Source: CAD feature listing. Evaluate the final solid. Frame: model axes, mm. Coordinates: 2 decimals unless noted, no trailing zeros. Loops run counter-clockwise (first coordinate to the right, second up) from the corner with the lowest first, then second, coordinate; pieces in that order, holes last.
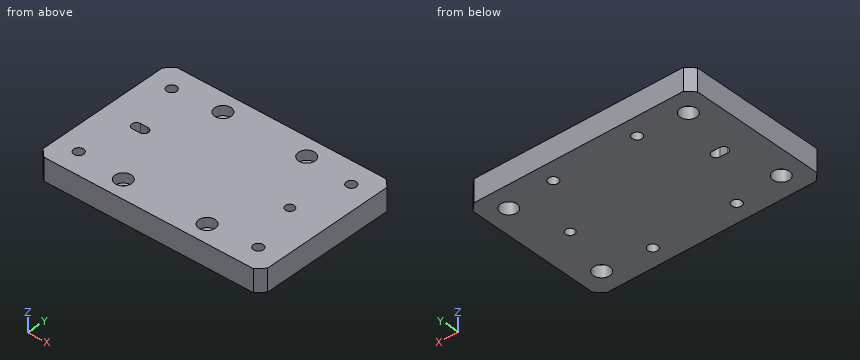
from build123d import *

# Parameters (mm, degrees)
SKETCH_1_W                   = 150
SKETCH_1_H                   = 100
EXTRUDE_1_DEPTH              = 7.5
HOLE_WIZARD_M6_1_D           = 6.6
HOLE_WIZARD_M6_1_CBORE_D     = 11
HOLE_WIZARD_M6_1_CBORE_DEPTH = 6.4
CHAMFER_1_SIZE               = 5
HOLE_WIZARD_M6_2_D           = 6.6
HOLE_WIZARD_M6_2_CBORE_D     = 11
HOLE_WIZARD_M6_2_CBORE_DEPTH = 8
MM_1_D                       = 6
CUT_EXTRUDE_1_DEPTH          = 92.378334412


with BuildPart() as part:
    # 草图1 → 凸台-拉伸1 (new, symmetric)
    with BuildSketch(Plane.XY):
        Rectangle(SKETCH_1_W, SKETCH_1_H)
    extrude(amount=EXTRUDE_1_DEPTH, both=True)

    # M6 六角凹头螺钉的柱形沉头孔1 (through all)
    with Locations(Plane.XY.offset(7.5)):
        with Locations((-28, -37.5), (-28, 37.5), (28, 37.5), (28, -37.5)):
            CounterBoreHole(HOLE_WIZARD_M6_1_D / 2, HOLE_WIZARD_M6_1_CBORE_D / 2, HOLE_WIZARD_M6_1_CBORE_DEPTH)

    # 倒角1
    chamfer_1_edges = [part.edges().sort_by_distance(p)[0] for p in [
        (75, -50, 0),
        (-75, -50, 0),
        (-75, 50, 0),
        (75, 50, 0),
    ]]
    chamfer(chamfer_1_edges, length=CHAMFER_1_SIZE)

    # M6 六角凹头螺钉的柱形沉头孔2 (through all)
    with Locations(Plane(origin=(0, 0, -7.5), x_dir=(-1, 0, 0), z_dir=(0, 0, -1))):
        with Locations((-60, -35), (-60, 35), (60, 35), (60, -35)):
            CounterBoreHole(HOLE_WIZARD_M6_2_D / 2, HOLE_WIZARD_M6_2_CBORE_D / 2, HOLE_WIZARD_M6_2_CBORE_DEPTH)

    # 大小mm 暗销孔1 (through all)
    with Locations(Plane(origin=(0, 0, -7.5), x_dir=(-1, 0, 0), z_dir=(0, 0, -1))):
        with Locations((50, 0), (-50, 0)):
            Hole(MM_1_D / 2)

    # 草图8 → 切除-拉伸1 (cut, through all)
    with BuildSketch(Plane(origin=(0, 0, -7.5), x_dir=(-1, 0, 0), z_dir=(0, 0, -1))):
        with BuildLine():
            Line((47.5, 3), (52.5, 3))
            ThreePointArc((52.5, 3), (55.5, 0), (52.5, -3))
            Line((52.5, -3), (47.5, -3))
            ThreePointArc((47.5, -3), (44.5, 0), (47.5, 3))
        make_face()
    extrude(amount=-CUT_EXTRUDE_1_DEPTH, mode=Mode.SUBTRACT)


solid = part.part
Q1. Line query: line 1 along Y through (x, z) = (28, 6.25); line 2 along Y through (x, z) = (60, 4.75); line 3 along Y through (x, z) = (50, 3.25). Output: solid intervals per line, ascending.
Q2. Contact query for flat-ended pins moving along their axis: pin 1 Ø1.5 at (x, y) = (58, 39) entering from -Z; pin 2 Ø7.5 at (x, y) = (-28, -37.5) entering from +Z. Output: stop coordinate, or through.
Q3. Section B-B, the plane x = 28. Return the cut outline in (y, z), plus the area to 3 significant figures.
Q4. Section A-A, the plane x = 50. Return the cut outline in (y, z).
Derived:
1. line 1: y = -50 to -43, -32 to 32, 43 to 50
1. line 2: y = -50 to -38.3, -31.7 to 31.7, 38.3 to 50
1. line 3: y = -50 to -3, 3 to 50
2. pin 1: stops at z = 0.5
2. pin 2: stops at z = 1.1
3. outline: (-50, -7.5) - (-40.8, -7.5) - (-40.8, 1.1) - (-43, 1.1) - (-43, 7.5) - (-50, 7.5) - close; (-34.2, -7.5) - (34.2, -7.5) - (34.2, 1.1) - (32, 1.1) - (32, 7.5) - (-32, 7.5) - (-32, 1.1) - (-34.2, 1.1) - close; (40.8, -7.5) - (50, -7.5) - (50, 7.5) - (43, 7.5) - (43, 1.1) - (40.8, 1.1) - close
3. area: 1,250 mm2
4. outline: (-50, -7.5) - (-3, -7.5) - (-3, 7.5) - (-50, 7.5) - close; (3, -7.5) - (50, -7.5) - (50, 7.5) - (3, 7.5) - close
